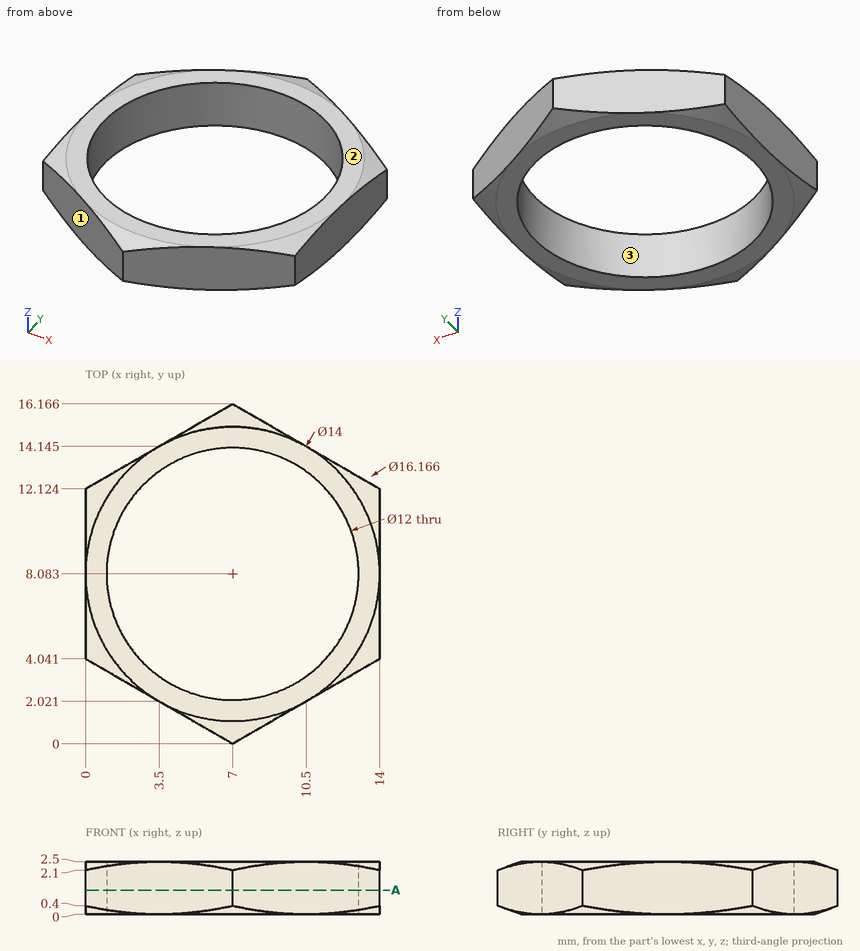
Study the drawing (mm; zero at the part's minimum x, y, z) and answer. Round coordinates to 2 decimals unless told otherwise and drop trailing zeros. Write each loop counter-clockwise with the first axis right and the second up, starting at its lowest first coordinate (ties: lowest second). Pieces come first, ordered by that corner, then holes.
1) Given pin 1 Ø1 at (y, z) = (13.5, 0.5) entering from -X (1 decimal); pin 2 Ø1 at (y, z) = (13.5, 0.5) entering from +X (1 decimal); pin 3 Ø1 at (x, z) = (2.5, 1) entering from +Y, each flat-ended and moving along its own axis, determine where each tip first touches the part or whether it passes through.
2) The mould has two halves that part along X. Classify the marked faces 1, 2 and 3: pulls with the +X half, pulls with the -X half, needs draft (parallel to the pull), parting line crosses it, or undercut.
3) Straight lines are drawn through the part: line 1 (X direction, y = 8.25, z = 1.9); line 2 (Y direction, x = 8.5, z = 1.4) (1 decimal); line 3 (X direction, y = 12.5, z = 0.5). For each, find the intervals that lie inside material, in ascending order.
4) A cutting plane is placed at A-A (z = 1.15). Give the vertices of the cut face in (x, y) (1 decimal).
Completed:
1. pin 1: stops at x = 1.5
1. pin 2: stops at x = 12.5
1. pin 3: stops at y = 13.86
2. face 1: pulls with the -X half
2. face 2: needs draft
2. face 3: undercut
3. line 1: x = 0 to 1, 13 to 14
3. line 2: y = 0.9 to 2.3, 13.9 to 15.3
3. line 3: x = 0.65 to 2.94, 11.06 to 13.35
4. outline: (0, 4) - (7, 0) - (14, 4) - (14, 12.1) - (7, 16.2) - (0, 12.1) - close; hole circle Ø12 at (7, 8.1)
